Here's how the part is built. I have some questions about the finished solid (model axes, mm). Give positions to 0.01 mm unless a question says otherwise; leave off trailing zeros. Loops run counter-clockwise (first coordinate to the right, second up) from the corner with the lowest first, then second, coordinate; pieces in that order, holes last.
Q1. Suppose I cut it at A-A (z = -120). List the corners of the cut face in (x, y) for me, and give its area (3 significant figures).
Q2. I need wall thicknesses on probe 1 along X at (y, z) = (9, -120). Which ranges of the line are inside material? Lowest first, please.
Q3. I'm going to push flat-ended pins straight in: P1, Ø10, axis at x = -60, z = -24.5, coming from the -Y side; P2, Ø17.5, axis at x = 220, z = -120, coming from the +Y side. Where does each tip first touch, or does it pass through?
Q4. Suppose I cut it at B-B (x = -220). List the corners of the cut face in (y, z) for me, and give its area (3 significant figures).
```python
from build123d import *

# Parameters (mm, degrees)
SKETCH1_W           = 600
SKETCH1_H           = 400
BOSS_EXTRUDE1_DEPTH = 20
SKETCH2_R           = 11
CUT_EXTRUDE1_DEPTH  = 20


with BuildPart() as part:
    # Sketch1 → Boss-Extrude1 (new body)
    with BuildSketch(Plane(origin=(0, 0, 0), x_dir=(1, 0, 0), z_dir=(0, 1, 0))):
        Rectangle(SKETCH1_W, SKETCH1_H)
    extrude(amount=BOSS_EXTRUDE1_DEPTH)

    # Sketch2 → Cut-Extrude1 (cut)
    with BuildSketch(Plane(origin=(0, 20, 0), x_dir=(1, 0, 0), z_dir=(0, 1, 0))):
        with Locations(Location((-220, 120, 0), (0, 0, 270))):
            Circle(SKETCH2_R)
        with Locations(Location((220, 120, 0), (0, 0, 90))):
            Circle(SKETCH2_R)
        with Locations(Location((220, -120, 0), (0, 0, 270))):
            Circle(SKETCH2_R)
        with Locations(Location((-220, -120, 0), (0, 0, 90))):
            Circle(SKETCH2_R)
    extrude(amount=-CUT_EXTRUDE1_DEPTH, mode=Mode.SUBTRACT)


solid = part.part
```
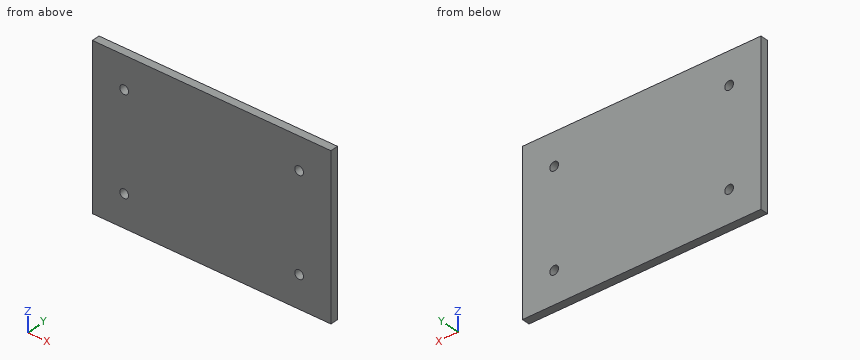
Solutions:
1. outline: (-300, 0) - (-231, 0) - (-231, 20) - (-300, 20) - close; (-209, 0) - (209, 0) - (209, 20) - (-209, 20) - close; (231, 0) - (300, 0) - (300, 20) - (231, 20) - close
1. area: 11,100 mm2
2. probe 1: x = -300 to -231, -209 to 209, 231 to 300
3. P1: stops at y = 0
3. P2: passes through
4. outline: (0, -200) - (20, -200) - (20, -131) - (0, -131) - close; (0, -109) - (20, -109) - (20, 109) - (0, 109) - close; (0, 131) - (20, 131) - (20, 200) - (0, 200) - close
4. area: 7,120 mm2
